```python
from build123d import *

# Parameters (mm, degrees)
SKETCH_3_R      = 19
EXTRUDE_2_DEPTH = 20


with BuildPart() as part:
    # 草图3 → 凸台-拉伸2 (new body)
    with BuildSketch(Plane.XY):
        with BuildLine():
            Line((0, 0), (-315, 0))
            Line((-315, 0), (-315, -90))
            ThreePointArc((-315, -90), (-309.142135624, -104.142135624), (-295, -110))
            Line((-295, -110), (-85.110940509, -110))
            ThreePointArc((-85.110940509, -110), (-80.159130316, -110.622704631), (-75.515671638, -112.452042418))
            Line((-75.515671638, -112.452042418), (8.890408484, -158.60550668))
            ThreePointArc((8.890408484, -158.60550668), (64.353360189, -147.492665271), (63.040388304, -90.942595767))
            Line((63.040388304, -90.942595767), (4.98164168, -24.925565564))
            ThreePointArc((4.98164168, -24.925565564), (1.286807242, -18.775729131), (0, -11.71765455))
            Line((0, -11.71765455), (0, 0))
        make_face()
        with Locations((30, -120)):
            Circle(SKETCH_3_R, mode=Mode.SUBTRACT)
        with BuildLine():
            Line((-270, -27.5), (-222, -27.5))
            ThreePointArc((-222, -27.5), (-204.5, -45), (-222, -62.5))
            Line((-222, -62.5), (-270, -62.5))
            ThreePointArc((-270, -62.5), (-287.5, -45), (-270, -27.5))
        make_face(mode=Mode.SUBTRACT)
        with BuildLine():
            Line((-160, -27.5), (-127, -27.5))
            ThreePointArc((-127, -27.5), (-109.5, -45), (-127, -62.5))
            Line((-127, -62.5), (-160, -62.5))
            ThreePointArc((-160, -62.5), (-177.5, -45), (-160, -27.5))
        make_face(mode=Mode.SUBTRACT)
    extrude(amount=EXTRUDE_2_DEPTH)


solid = part.part
```
Verification items for the finished model (mm, model axes). A direction names the side the tool comes from. Coordinates: 2 decimals unless noted, no trailing zeros. Order: outer loops, then holes, each group sorted by start corner. A loop starts at its lowest first (then second) coordinate and runs counter-clockwise, first axis right, second up. Notation, with made-up numbers: (46, 36) -> (63, 36) arc R30 ccw to (63, 70) -> close; hole circle Ø6 at (30.25, -2.5). An arc over 180 degrees is marked (long way). Answer as CSV lines item,"result". Start each with the question number.
1) Cross-section at D-D, the plane y = -45. Record the boundary of the cut face in (x, z).
2) Release check for a two-part mould opening along X. For faces 1 (the face through (-287.496, -45.385, 9.86)), 2 (the face through (34.42, -58.4, 9.86)), 3 (the face through (-80.227, -110.605, 9.86)) record: released by +X, released by -X, zero draft, split by the parting line, or undercut.
3) Set-up check for faces 4 (the face through (0, -6, 10)), 5 (the face through (-123, -63, 20)), 6 (the face through (-109.504, -44.615, 9.86)): record each of +Z, -Z, +X, -X, +Y, -Y from which the full face is reachable in a straight line by a thin tool's end or side.
4) Cross-section at A-A, the plane y = -128. Record the boundary of the cut face in (x, z).
5) Gauge pin test, flat ends, axial feed: pin 1 Ø6 at (x, z) = (-203, 12) entering from -Y; pin 2 Ø6 at (y, z) = (-113, 7.5) entering from +X; pin 3 Ø23 at (x, y) = (30, -120) entering from -Z (3 decimals); pin 4 Ø2 at (x, z) = (-81.5, 6.5) entering from -Y. Record the tip position at first contact, or that the pin passes through.
6) Cross-section at B-B, the plane z = 13. Record the boundary of the cut face in (x, y).
7) Cross-section at C-C, the plane x = 30. Record the boundary of the cut face in (y, z).
8) Material ranges on L1, parallel to Y at x = -145, z = 13.75; L2, parallel to X at y = -9, z = 7.75; L3, parallel to Y at x = -180, z = 18.25, recorded low to high. Write a range as [from, to].
Conclusion:
1,outline,"(-315, 0) -> (-287.5, 0) -> (-287.5, 20) -> (-315, 20) -> close; (-204.5, 0) -> (-177.5, 0) -> (-177.5, 20) -> (-204.5, 20) -> close; (-109.5, 0) -> (22.64, 0) -> (22.64, 20) -> (-109.5, 20) -> close"
2,face 1,"undercut"
2,face 2,"released by +X"
2,face 3,"released by -X"
3,face 4,"+Z, -Z, +X, +Y"
3,face 5,"+Z, +X, -X, +Y, -Y"
3,face 6,"+Z, -Z"
4,outline,"(-47.08, 0) -> (12.77, 0) -> (12.77, 20) -> (-47.08, 20) -> close; (47.23, 0) -> (73.27, 0) -> (73.27, 20) -> (47.23, 20) -> close"
5,pin 1,"stops at y = -110"
5,pin 2,"stops at x = 73.82"
5,pin 3,"passes through"
5,pin 4,"stops at y = -110.54"
6,outline,"(-315, -90) arc R20 ccw to (-295, -110) -> (-85.11, -110) arc R20 cw to (-75.52, -112.45) -> (8.89, -158.61) arc R44 ccw to (63.04, -90.94) -> (4.98, -24.93) arc R20 cw to (0, -11.72) -> (0, 0) -> (-315, 0) -> close; hole (-270, -62.5) -> (-222, -62.5) arc R17.5 ccw to (-222, -27.5) -> (-270, -27.5) arc R17.5 ccw to start; hole (-160, -62.5) -> (-127, -62.5) arc R17.5 ccw to (-127, -27.5) -> (-160, -27.5) arc R17.5 ccw to start; hole circle Ø38 at (30, -120)"
7,outline,"(-164, 0) -> (-139, 0) -> (-139, 20) -> (-164, 20) -> close; (-101, 0) -> (-53.37, 0) -> (-53.37, 20) -> (-101, 20) -> close"
8,L1,"y = [-110, -62.5], [-27.5, 0]"
8,L2,"x = [-315, 0]"
8,L3,"y = [-110, 0]"
